from build123d import *

# Parameters (mm, degrees)
BOSS_EXTRUDE1_DEPTH = 11


with BuildPart() as part:
    # Sketch1 → Boss-Extrude1 (new body)
    with BuildSketch(Plane.XY):
        with BuildLine():
            Line((-18.363387922, 23.381087781), (-18.363387922, 75.858020773))
            ThreePointArc((-18.363387922, 75.858020773), (-39.363387922, 96.858020773), (-60.363387922, 75.858020773))
            Line((-60.363387922, 75.858020773), (-60.363387922, 22.707373273))
            ThreePointArc((-60.363387922, 22.707373273), (-42.401334766, -20.656859064), (0.962897571, -38.618912219))
            Line((0.962897571, -38.618912219), (179.480864488, -38.618912219))
            ThreePointArc((179.480864488, -38.618912219), (200.480864488, -17.618912219), (179.480864488, 3.381087781))
            Line((179.480864488, 3.381087781), (1.636612078, 3.381087781))
            ThreePointArc((1.636612078, 3.381087781), (-12.505523546, 9.238952157), (-18.363387922, 23.381087781))
        make_face()
        with BuildLine():
            Line((-55.363387922, 75.858020773), (-55.363387922, 22.707373273))
            ThreePointArc((-55.363387922, 22.707373273), (-38.86580086, -17.121325158), (0.962897571, -33.618912219))
            Line((0.962897571, -33.618912219), (179.480864488, -33.618912219))
            ThreePointArc((179.480864488, -33.618912219), (195.480864488, -17.618912219), (179.480864488, -1.618912219))
            Line((179.480864488, -1.618912219), (1.636612078, -1.618912219))
            ThreePointArc((1.636612078, -1.618912219), (-16.041057452, 5.703418251), (-23.363387922, 23.381087781))
            Line((-23.363387922, 23.381087781), (-23.363387922, 75.858020773))
            ThreePointArc((-23.363387922, 75.858020773), (-39.363387922, 91.858020773), (-55.363387922, 75.858020773))
        make_face(mode=Mode.SUBTRACT)
    extrude(amount=-BOSS_EXTRUDE1_DEPTH)


solid = part.part
Read the model definition and answer for the solid it produces. Units are mm, in the model's axes. A direction names the side the tool comes from. Give positions to 0.01 mm unless a question says otherwise; leave off trailing zeros. Write each loop counter-clockwise with the first axis right and the second up, starting at its lowest first coordinate (ties: lowest second). Pieces come first, ordered by that corner, then holes. Notation, with made-up numbers: (-35, 89.25) - (-10, 89.25) arc R29 cw to (-10, 120.25) - close; hole circle Ø8 at (89.5, 3). An arc over 180 degrees is marked (long way). Answer in a Markdown table with one row per item. Add a question column.
Item 1: Find the intervals of material crossed by L1, parallel to Y at x = 64.5, z = -9.25; L2, parallel to X at y = 74.5, z = -4.25; L3, parallel to X at y = 81, z = -1, in increasing order.
Item 2: Section B-B, the plane x = 149 is taken. Write down the section's boundary in (y, z), and give its area (3 significant figures).
Item 3: Flat-ended cylindrical pins translate along their axes: P1, Ø5, axis at x = 124.5, y = -4.5, coming from the -Z side; P2, Ø5.5, axis at x = 130, z = -5, coming from the +Y side. Find the tip coordinate at first contact, or state that the pin passes through.
Item 4: Section A-A, the plane z = -2.5 is taken. Write down the section's boundary in (x, y).
Item 5: A tool of negligible diameter and unlimited length cuts with its end or side. For faces 5 (the face through (-60.363, 50, -5)), 6 (the face through (-39.012, 91.854, -5.423)), 7 (the face through (92, 3.381, -5)), from which of +Z, -Z, +X, -X, +Y, -Y can it reach the whole face along a straight path? Write none if from no direction.
Item 6: Determine the mould class of faces 1 (the face through (89, -33.619, -5)), 2 (the face through (89, -38.619, -5)), 3 (the face through (40, -1, 0)), 4 (the face through (200.476, -18.081, -5.423)) for opening direction Y: pulls with the +Y half, pulls with the -Y half, needs draft (parallel to the pull), parting line crosses it, or undercut.
Item 7: Section C-C, the plane y = 34 is taken. Write down the section's boundary in (x, z), and give its area (3 significant figures).
Recorded:
| question | item | result |
|---|---|---|
| 1 | L1 | y = -38.62 to -33.62, -1.62 to 3.38 |
| 1 | L2 | x = -60.36 to -55.36, -23.36 to -18.36 |
| 1 | L3 | x = -59.72 to -54.51, -24.21 to -19 |
| 2 | outline | (-38.62, -11) - (-33.62, -11) - (-33.62, 0) - (-38.62, 0) - close; (-1.62, -11) - (3.38, -11) - (3.38, 0) - (-1.62, 0) - close |
| 2 | area | 110 mm2 |
| 3 | P1 | passes through |
| 3 | P2 | stops at y = 3.38 |
| 4 | outline | (-60.36, 22.71) arc R61.33 ccw to (0.96, -38.62) - (179.48, -38.62) arc R21 ccw to (179.48, 3.38) - (1.64, 3.38) arc R20 cw to (-18.36, 23.38) - (-18.36, 75.86) arc R21 ccw to (-60.36, 75.86) - close; hole (-55.36, 22.71) arc R56.33 ccw to (0.96, -33.62) - (179.48, -33.62) arc R16 ccw to (179.48, -1.62) - (1.64, -1.62) arc R25 cw to (-23.36, 23.38) - (-23.36, 75.86) arc R16 ccw to (-55.36, 75.86) - close |
| 5 | face 5 | +Z, -Z, -X, +Y, -Y |
| 5 | face 6 | +Z, -Z |
| 5 | face 7 | +Z, -Z, +X, +Y |
| 6 | face 1 | undercut |
| 6 | face 2 | pulls with the -Y half |
| 6 | face 3 | needs draft |
| 6 | face 4 | parting line crosses it |
| 7 | outline | (-60.36, -11) - (-55.36, -11) - (-55.36, 0) - (-60.36, 0) - close; (-23.36, -11) - (-18.36, -11) - (-18.36, 0) - (-23.36, 0) - close |
| 7 | area | 110 mm2 |
